Can you work these out from the model? Positions are in its coordinate system, mm. A direction names the side the tool comes from. Give positions to 0.01 mm unless a question says otherwise; leave off trailing zeros. Order: outer loops, then holes, each group sorted by start corner. A loop starts at its lowest first (then second) coordinate and runs counter-clockwise, first axis right, second up. Notation, with made-up numbers: M 83.25,14 L 107.25,14 A33 ccw 107.25,46 Z; hole C -12.5,73.25 d2. An arc over 180 degrees is marked long. Answer as a JSON object with one key per item and string values.
```python
from build123d import *

# Parameters (mm, degrees)
BOSS_EXTRUDE1_DEPTH = 60
SKETCH2_R           = 13
CUT_EXTRUDE1_DEPTH  = 87
SKETCH3_R           = 11
CUT_EXTRUDE2_DEPTH  = 87
CUT_EXTRUDE3_DEPTH  = 15


with BuildPart() as part:
    # Sketch1 → Boss-Extrude1 (new, symmetric)
    with BuildSketch(Plane.XY):
        with BuildLine():
            Line((-200, 0), (200, 0))
            Line((200, 0), (200, 40))
            Line((200, 40), (127.5, 40))
            ThreePointArc((127.5, 40), (120.428932188, 42.928932188), (117.5, 50))
            Line((117.5, 50), (117.5, 205))
            ThreePointArc((117.5, 205), (118.964466094, 208.535533906), (122.5, 210))
            Line((122.5, 210), (175, 210))
            Line((175, 210), (175, 235))
            Line((175, 235), (92, 235))
            Line((92, 235), (90, 233))
            Line((90, 233), (90, 57))
            ThreePointArc((90, 57), (87.071067812, 49.928932188), (80, 47))
            Line((80, 47), (-80, 47))
            ThreePointArc((-80, 47), (-87.071067812, 49.928932188), (-90, 57))
            Line((-90, 57), (-90, 233))
            Line((-90, 233), (-92, 235))
            Line((-92, 235), (-175, 235))
            Line((-175, 235), (-175, 210))
            Line((-175, 210), (-122.5, 210))
            ThreePointArc((-122.5, 210), (-118.964466094, 208.535533906), (-117.5, 205))
            Line((-117.5, 205), (-117.5, 50))
            ThreePointArc((-117.5, 50), (-120.428932188, 42.928932188), (-127.5, 40))
            Line((-127.5, 40), (-200, 40))
            Line((-200, 40), (-200, 0))
        make_face()
    extrude(amount=BOSS_EXTRUDE1_DEPTH, both=True)

    # Sketch2 → Cut-Extrude1 (cut)
    with BuildSketch(Plane.XZ):
        with Locations(Location((-160, 0, 0), (0, 0, 270))):
            Circle(SKETCH2_R)
        with Locations(Location((160, 0, 0), (0, 0, 270))):
            Circle(SKETCH2_R)
    extrude(amount=-CUT_EXTRUDE1_DEPTH, mode=Mode.SUBTRACT)

    # Sketch3 → Cut-Extrude2 (cut)
    with BuildSketch(Plane(origin=(0, 235, 0), x_dir=(1, 0, 0), z_dir=(0, 1, 0))):
        with Locations(Location((-145, 0, 0), (0, 0, 270))):
            Circle(SKETCH3_R)
        with Locations(Location((145, 0, 0), (0, 0, 180))):
            Circle(SKETCH3_R)
    extrude(amount=-CUT_EXTRUDE2_DEPTH, mode=Mode.SUBTRACT)

    # Sketch4 → Cut-Extrude3 (cut)
    with BuildSketch(Plane(origin=(0, 0, -60), x_dir=(-1, 0, 0), z_dir=(0, 0, -1))):
        with BuildLine():
            Line((-105, 140), (-105, 340))
            Line((-105, 340), (105, 340))
            Line((105, 340), (105, 140))
            ThreePointArc((105, 140), (0, 35), (-105, 140))
        make_face()
    extrude(amount=-CUT_EXTRUDE3_DEPTH, mode=Mode.SUBTRACT)


solid = part.part
```
1) I want a section at A-A on x = 160. Write out the boundary of the cut face in (y, z).
Results found:
{"outline": "M 0,-60 L 40,-60 L 40,-13 L 0,-13 Z; M 0,13 L 40,13 L 40,60 L 0,60 Z; M 210,-60 L 235,-60 L 235,60 L 210,60 Z"}
2) I'm going to push flat-ended pins straight in: pin 1 Ø7.5 at (x, y) = (97.5, 177) entering from -Z; pin 2 Ø8 at (x, z) = (8, 41.5) entering from +Y; pin 3 Ø1 at (y, z) = (190, 38) entering from -X. Where does each tip first touch, or does it pass through?
Results found:
{"pin 1": "stops at z = -45", "pin 2": "stops at y = 47", "pin 3": "stops at x = -117.5"}
3) I want a section at C-C on z = 20.5. Write out the boundary of the cut face in (x, y).
Results found:
{"outline": "M -200,0 L 200,0 L 200,40 L 127.5,40 A10 cw 117.5,50 L 117.5,205 A5 cw 122.5,210 L 175,210 L 175,235 L 92,235 L 90,233 L 90,57 A10 cw 80,47 L -80,47 A10 cw -90,57 L -90,233 L -92,235 L -175,235 L -175,210 L -122.5,210 A5 cw -117.5,205 L -117.5,50 A10 cw -127.5,40 L -200,40 Z"}
4) I want a section at D-D on z = 0. Count the separate pieces of the cut face and the enclosed holes in it, and give its area (3 significant figures).
Results found:
{"separate pieces": "5", "enclosed holes": "0", "area": "27,800 mm²"}
5) I need wall thicknesses on L1, parallel to X at y = 25, z = 0; L2, parallel to Y at x = -132, z = -32.5; L3, parallel to X at y = 176, z = 23.5. Which ranges of each line are inside material? Lowest first, please.
Results found:
{"L1": "x = -200 to -173, -147 to 147, 173 to 200", "L2": "y = 0 to 40, 210 to 235", "L3": "x = -117.5 to -90, 90 to 117.5"}
6) Thinking about a two-plate mould opening in X: for faces 5 (the face through (-163, 40, 14)), 6 (the face through (-175, 223, 1)), 7 (the face through (101.074, 111.555, -52.605)), which applies, pulls with the +X half, pulls with the -X half, needs draft (parallel to the pull), parting line crosses it, or undercut?
Results found:
{"face 5": "needs draft", "face 6": "pulls with the -X half", "face 7": "undercut"}
7) I want a section at B-B on y = 173.5. Write out the boundary of the cut face in (x, z), and give its area (3 significant figures).
Results found:
{"outline": "M -117.5,-60 L -105,-60 L -105,-45 L -90,-45 L -90,60 L -117.5,60 Z; M 90,-45 L 105,-45 L 105,-60 L 117.5,-60 L 117.5,60 L 90,60 Z", "area": "6,150 mm²"}
8) For faces 1 (the face through (-161, 210, 1)), 2 (the face through (1, 47, 1)), 3 (the face through (156, 223, 0)), 4 (the face through (-1, 42, -45)), which set-ups out of +Z, -Z, +X, -X, +Y, -Y let a thin tool reach every point of the face, with its end or its side?
Results found:
{"face 1": "+Z, -Z, -X", "face 2": "+Z, -Z, +Y", "face 3": "+Y", "face 4": "-Z, +Y"}
